Source: three-view drawing plus pictorial views. Frame: mm from the lowest corner of the part. A direction names the side the tool comes from. Round coordinates to 2 decimals unless told otherwise and drop trailing zeros. Loops run counter-clockwise (first coordinate to the right, second up) from the corner with the lowest first, then second, coordinate; pieces in that order, holes last. Notation, with made-up numbers: (-12.5, 15) -> (25.5, 15) arc R15 cw to (25.5, 33) -> close; hole circle Ø3 at (27, 86.5). An arc over 180 degrees is marked (long way). Return JSON: item names as keys, results as strings. Group by question number.
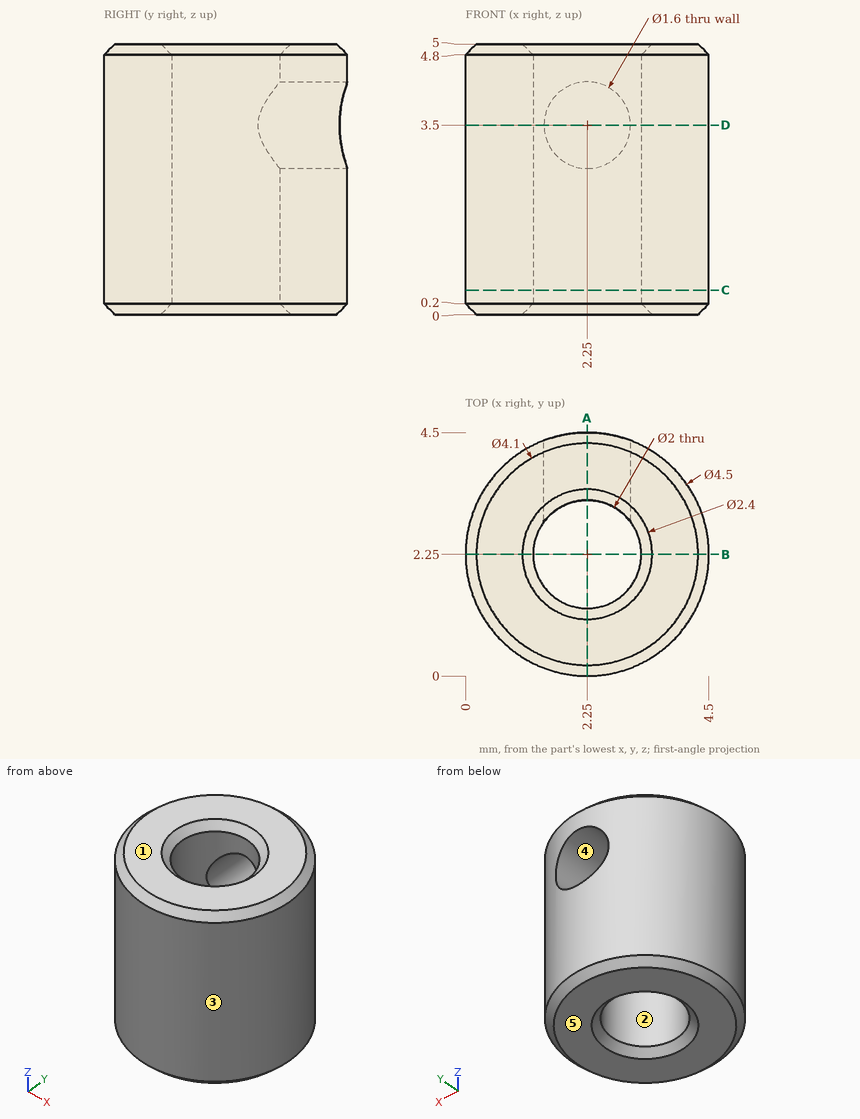
(1) Pin query (flat end, axial travel): pin 1 (1.2 mm diameter, centred on x = 2.25, y = 2.25, fed in from -Z); pin 2 (2 mm diameter, centred on y = 3.5, z = 4, fed in from -X); pin 3 (1.5 mm diameter, centred on x = 0.5, z = 4, fed in from +Y); pin 4 (1.5 mm diameter, centred on x = 1, y = 0.5, fed in from -Z). Return the tip coordinate at first contact, or that it passes through.
(2) Cut plane D-D (z = 3.5). Return loops of the section in (x, y).
(3) Set-up query: the marked faces 4 and 5. Return all of +Z, -Z, +X, -X, +Y, -Y with unobstructed straight access to the full face (end or side cutting, diameter ignored); none if empty.
(4) Mould query, pull axis Y, two halves, no side actions, for the marked faces 1, 2 and 3. Classes: released by +Y, released by -Y, zero draft, split by the parting line, or undercut.
(5) Cut plane B-B (y = 2.25). Return loops of the section in (x, z), and give its area (3 significant figures).
(6) Cut plane A-A (x = 2.25). Return loops of the section in (y, z), and give its area (3 significant figures).
(7) Cut plane C-C (z = 0.45). Return loops of the section in (x, y), and give its area (3 significant figures).
(8) Ray query, line 1 (Y direction, x = 2.25, z = 1.65); line 2 (X direction, y = 3.2, z = 3.5); line 3 (X direction, y = 1.5, z = 2.9). Return the intervals inside material, ascending.
Answers follow:
{
 "1": {"pin 1": "through", "pin 2": "x = 0.01", "pin 3": "y = 4.27", "pin 4": "z = 0"},
 "2": {"outline": "(1.45, 2.85) -> (1.45, 4.35) arc R2.25 ccw (long way) to (3.05, 4.35) -> (3.05, 2.85) arc R1 cw (long way) to start"},
 "3": {"face 4": "+Y", "face 5": "-Z, +X, -X, +Y, -Y"},
 "4": {"face 1": "zero draft", "face 2": "undercut", "face 3": "split by the parting line"},
 "5": {"outline": "(0, 0.2) -> (0.2, 0) -> (1.05, 0) -> (1.25, 0.2) -> (1.25, 4.8) -> (1.05, 5) -> (0.2, 5) -> (0, 4.8) -> close; (3.25, 0.2) -> (3.45, 0) -> (4.3, 0) -> (4.5, 0.2) -> (4.5, 4.8) -> (4.3, 5) -> (3.45, 5) -> (3.25, 4.8) -> close", "area": "12.3 mm^2"},
 "6": {"outline": "(0, 0.2) -> (0.2, 0) -> (1.05, 0) -> (1.25, 0.2) -> (1.25, 4.8) -> (1.05, 5) -> (0.2, 5) -> (0, 4.8) -> close; (3.25, 0.2) -> (3.45, 0) -> (4.3, 0) -> (4.5, 0.2) -> (4.5, 2.7) -> (3.25, 2.7) -> close; (3.25, 4.3) -> (4.5, 4.3) -> (4.5, 4.8) -> (4.3, 5) -> (3.45, 5) -> (3.25, 4.8) -> close", "area": "10.3 mm^2"},
 "7": {"outline": "circle Ø4.5 at (2.25, 2.25); hole circle Ø2 at (2.25, 2.25)", "area": "12.8 mm^2"},
 "8": {"line 1": "0 to 1.25, 3.25 to 4.5", "line 2": "0.21 to 1.45, 3.05 to 4.29", "line 3": "0.13 to 1.59, 2.91 to 4.37"}
}
